CAD build for the part. Positions are in the model's coordinates, mm. Give positions to 0.01 mm unless a question says otherwise; leave off trailing zeros. Loops run counter-clockwise (first coordinate to the right, second up) from the corner with the lowest first, then second, coordinate; pieces in that order, holes last. Notation, with made-up numbers: (77, -2) -> (118, -2) arc R29 cw to (118, 34) -> close; hole circle Ø1 at (6, 87). An arc over 180 degrees is marked (long way). Use one line per item in the form item = value.
```python
from build123d import *

# Parameters (mm, degrees)
SKETCH1_W           = 129
SKETCH1_H           = 30
BOSS_EXTRUDE1_DEPTH = 5
CUT_EXTRUDE1_REACH  = 68.41
SKETCH3_R           = 4
CHAMFER1_SIZE       = 1


with BuildPart() as part:
    # Sketch1 → Boss-Extrude1 (new body)
    with BuildSketch(Plane(origin=(0, 0, 0), x_dir=(1, 0, 0), z_dir=(0, 1, 0))):
        Rectangle(SKETCH1_W, SKETCH1_H)
    extrude(amount=BOSS_EXTRUDE1_DEPTH)

    # Sketch3 → Cut-Extrude1 (cut, up to next)
    with BuildSketch(Plane(origin=(0, 5, 0), x_dir=(1, 0, 0), z_dir=(0, 1, 0)), mode=Mode.PRIVATE) as cut_extrude1_sk1:
        with Locations(Location((0, 0, 0), (0, 0, 270))):
            Circle(SKETCH3_R)
    cut_extrude1_tool1 = extrude(cut_extrude1_sk1.sketch, amount=-CUT_EXTRUDE1_REACH, mode=Mode.PRIVATE) & part.part
    add(cut_extrude1_tool1.solids().sort_by_distance((0, 5, 0))[0], mode=Mode.SUBTRACT)

    # Chamfer1
    chamfer1_edges = [part.edges().sort_by_distance(p)[0] for p in [
        (-64.5, 5, 0),
        (0, 5, 15),
        (64.5, 5, 0),
        (0, 5, -15),
    ]]
    chamfer(chamfer1_edges, length=CHAMFER1_SIZE)


solid = part.part
```
1. Mould opens along Z. For faces 1 (the cylindrical face through (-3.905, 2.535, -0.867)), 2 (the flat face through (-1, 0, -7)), 3 (the flat face through (-1, 2, -15)) say: pulls with the +Z half, pulls with the -Z half, needs draft (parallel to the pull), parting line crosses it, or undercut.
Result sheet:
face_1 = undercut
face_2 = needs draft
face_3 = pulls with the -Z half
2. Cut at A-A, the plane x = 0. Write the cut outline in (y, z), then the cut area to 3 significant figures.
Result sheet:
outline = (0, -15) -> (4, -15) -> (5, -14) -> (5, -4) -> (0, -4) -> close; (0, 4) -> (5, 4) -> (5, 14) -> (4, 15) -> (0, 15) -> close
area = 109 mm^2
3. Cut at B-B, the plane z = 0. Write the cut outline in (x, y), then the cut area to 3 significant figures.
Result sheet:
outline = (-64.5, 0) -> (-4, 0) -> (-4, 5) -> (-63.5, 5) -> (-64.5, 4) -> close; (4, 0) -> (64.5, 0) -> (64.5, 4) -> (63.5, 5) -> (4, 5) -> close
area = 604 mm^2
4. Drop a flat-ended pin along its axis: P1, Ø4, axis at x = 9.5, z = 4.5, coming from the -Y side. Give the stop position or say it passes through.
Result sheet:
P1 = 0
5. Drill centre lines: line 1 (X direction, y = 1.3, z = 0); line 2 (X direction, y = 4.45, z = 3); line 3 (Z direction, x = -3.5, y = 1.3). Where is each one in solid material? Low to high.
Result sheet:
line_1 = -64.5 to -4, 4 to 64.5
line_2 = -64.05 to -2.65, 2.65 to 64.05
line_3 = -15 to -1.94, 1.94 to 15
